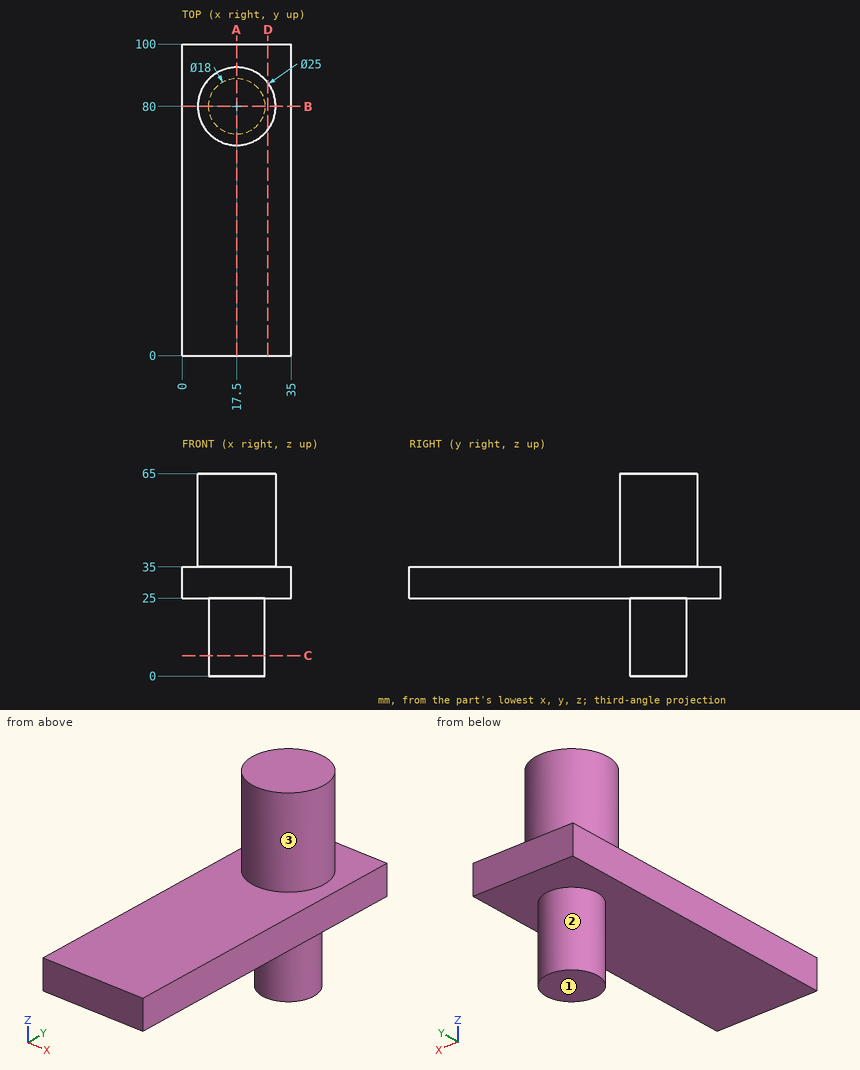
Print and shaded views of the part. All mm, measured from the part's lowest x, y and z. A direction names the side the tool comes from. Round coordinates to 2 decimals unless told otherwise and drop trailing zeros. Write each loop counter-clockwise with the first axis right and the second up, starting at its lowest first coordinate (ties: lowest second). Pieces come first, ordered by that corner, then holes. Notation, with made-up numbers: (70.25, 82.5) - (117.25, 82.5) arc R23 ccw to (117.25, 114.5) - close; hole circle Ø11 at (-13, 18). An arc over 180 degrees is marked (long way). Use CSV: the item, a comma, the result in double quotes. Start each with the question number.
Item 1: Pin check, flat tips, straight feed: P1, Ø5, axis at x = 24.5, y = 51.5, coming from the +Z side; P2, Ø8, axis at y = 35.5, z = 18.5, coming from the -X side. Stop position of each tip, or through.
Item 2: Drill centre lines: L1, parallel to Z at x = 10, y = 41; L2, parallel to Z at x = 10.5, y = 86; L3, parallel to Y at x = 18, z = 42. Where is each one in solid material? Low to high. Write a range as [from, to].
Item 3: Band-saw the part on C-C (z = 6.5). Write the cut outline in (x, y).
Item 4: Band-saw the part on D-D (x = 27.5). Write the cut outline in (y, z).
Item 5: Band-saw the part on B-B (y = 80). Write the cut outline in (x, z).
Item 6: Band-saw the part on A-A (x = 17.5). Write the cut outline in (y, z), and give its area (3 significant figures).
Item 7: Tool access for the marked faces 1, 2 and 3: list every direction of +Z, -Z, +X, -X, +Y, -Y with a clear straight run to the whole face (end or side of a thin tool).
Checked values:
1,P1,"stops at z = 35"
1,P2,"passes through"
2,L1,"z = [25, 35]"
2,L2,"z = [25, 65]"
2,L3,"y = [67.51, 92.49]"
3,outline,"circle Ø18 at (17.5, 80)"
4,outline,"(0, 25) - (100, 25) - (100, 35) - (87.5, 35) - (87.5, 65) - (72.5, 65) - (72.5, 35) - (0, 35) - close"
5,outline,"(0, 25) - (8.5, 25) - (8.5, 0) - (26.5, 0) - (26.5, 25) - (35, 25) - (35, 35) - (30, 35) - (30, 65) - (5, 65) - (5, 35) - (0, 35) - close"
6,outline,"(0, 25) - (71, 25) - (71, 0) - (89, 0) - (89, 25) - (100, 25) - (100, 35) - (92.5, 35) - (92.5, 65) - (67.5, 65) - (67.5, 35) - (0, 35) - close"
6,area,"2,200 mm²"
7,face 1,"-Z, +X, -X, +Y, -Y"
7,face 2,"-Z"
7,face 3,"+Z"
